```python
from build123d import *

# Parameters (mm, degrees)
EXTRUDE_1_DEPTH      = 5
EXTRUDE_1_DEPTH_BACK = 5


with BuildPart() as part:
    # 草图2 → 旋转1 (revolve)
    with BuildSketch(Plane.XY, mode=Mode.PRIVATE) as revolve_1_sk:
        with BuildLine():
            Line((6.5, 21.057334971), (6.5, 4.5))
            Line((6.5, 4.5), (5.633974596, 4))
            Line((5.633974596, 4), (0, 4))
            Line((0, 4), (0, 22.97165153))
            ThreePointArc((0, 22.97165153), (2.770599147, 22.808562355), (5.502930419, 22.321547438))
            ThreePointArc((5.502930419, 22.321547438), (6.220737367, 21.862378589), (6.5, 21.057334971))
        make_face()
    revolve(revolve_1_sk.sketch.rotate(Axis((0, 4, 0), (0, 1, 0)), 270), axis=Axis((0, 4, 0), (0, 1, 0)))

    # 草图1 → 凸台-拉伸1 (add, two sides: drawn at the far end of the back side and taken through both)
    with BuildSketch(Plane.XY.offset(-EXTRUDE_1_DEPTH_BACK)):
        with BuildLine():
            Line((-3.333333333, 5.5), (3.25, 5.5))
            Line((3.25, 5.5), (3.25, 10.326555972))
            ThreePointArc((3.25, 10.326555972), (4.489879958, 13.979124546), (7.697085729, 16.12211093))
            ThreePointArc((7.697085729, 16.12211093), (17.943826668, 18.039495945), (27.776457135, 21.502362282))
            ThreePointArc((27.776457135, 21.502362282), (29.380060021, 22.573855474), (30, 24.400139761))
            Line((30, 24.400139761), (30, 26))
            ThreePointArc((30, 26), (29.121320344, 28.121320344), (27, 29))
            Line((27, 29), (25.932943889, 29))
            Line((25.932943889, 29), (-3.333333333, 21.158124653))
            Line((-3.333333333, 21.158124653), (-3.333333333, 5.5))
        make_face()
    extrude(amount=EXTRUDE_1_DEPTH + EXTRUDE_1_DEPTH_BACK)

    # 草图3 → 切除-旋转1 (revolve, cut)
    with BuildSketch(Plane.XY, mode=Mode.PRIVATE) as cut_revolve_1_sk:
        Polygon((0, 28.156296), (4, 28.156296), (4, 17.156296), (5, 17.156296), (5, -2.643704), (0, -2.643704), align=None)
    revolve(cut_revolve_1_sk.sketch.rotate(Axis((0, -2.643704, 0), (0, 1, 0)), 270), axis=Axis((0, -2.643704, 0), (0, 1, 0)), mode=Mode.SUBTRACT)


solid = part.part
```
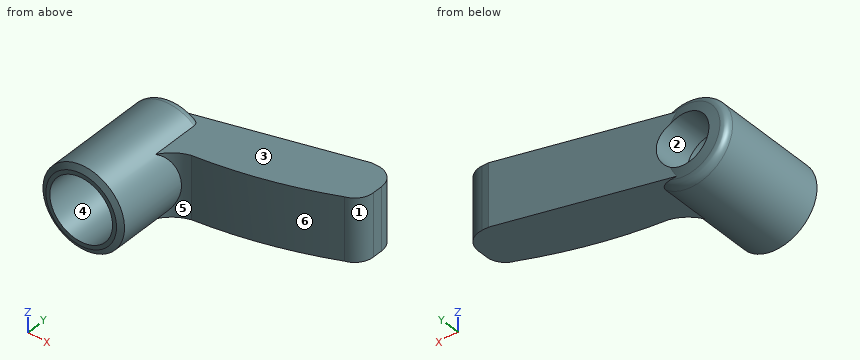
Input: part model. Units: mm. Frame: model coordinates. Face numbers are marked on the shaded views. A direction names the side the tool comes from. Coordinates: 2 decimals unless noted, no trailing zeros. Loops run counter-clockwise (first coordinate to the right, second up) from the corner with the lowest first, then second, coordinate; pieces in that order, holes last. Notation, with made-up numbers: (-40, 80) -> (-9, 80) arc R20 ccw to (-9, 93) -> close; hole circle Ø11 at (33.5, 75.5). An arc over 180 degrees is marked (long way). Use a Markdown table: item, result.
1) Cut plane C-C (z = 0). Return the cut outline in (x, y), then the cut area to 3 significant figures.
Results found:
| item | result |
|---|---|
| outline | (-6.5, 4.5) -> (-5.63, 4) -> (-5, 4) -> (-5, 17.16) -> (-4, 17.16) -> (-4, 22.63) arc R23.62 ccw to (-5.5, 22.32) arc R1.3 ccw to (-6.5, 21.06) -> close; (4, 17.16) -> (5, 17.16) -> (5, 4) -> (5.63, 4) -> (6.5, 4.5) -> (6.5, 15.66) arc R6 cw to (7.7, 16.12) arc R67.92 ccw to (27.78, 21.5) arc R3 ccw to (30, 24.4) -> (30, 26) arc R3 ccw to (27, 29) -> (25.93, 29) -> (4, 23.12) -> close |
| area | 261 mm2 |
2) Cut plane B-B (y = 10.5). Return the cut outline in (x, z).
Results found:
| item | result |
|---|---|
| outline | circle Ø13 at (0, 0); hole circle Ø10 at (0, 0) |
3) Pull-direction query (Z, two-part tool) for the marked faces 1, 2 and 3; classes: released by +Z, released by -Z, zero draft, split by the parting line, or undercut.
Results found:
| item | result |
|---|---|
| face 1 | zero draft |
| face 2 | undercut |
| face 3 | released by +Z |
4) Cut plane D-D (y = 14.25). Return the cut outline in (x, z), then the cut area to 3 significant figures.
Results found:
| item | result |
|---|---|
| outline | (4.15, -5) -> (4.71, -5) -> (4.71, -4.48) arc R6.5 ccw to (4.71, 4.48) -> (4.71, 5) -> (4.15, 5) arc R6.5 ccw (long way) to start; hole circle Ø10 at (0, 0) |
| area | 54.5 mm2 |
5) Cut plane A-A (x = 0). Return the cut outline in (y, z).
Results found:
| item | result |
|---|---|
| outline | (4, -5.63) -> (4.5, -6.5) -> (21.06, -6.5) arc R1.3 ccw to (22.32, -5.5) arc R23.62 ccw to (22.63, -4) -> (17.16, -4) -> (17.16, -5) -> (4, -5) -> close; (4, 5) -> (17.16, 5) -> (17.16, 4) -> (22.63, 4) arc R23.62 ccw to (22.32, 5.5) arc R1.3 ccw to (21.06, 6.5) -> (4.5, 6.5) -> (4, 5.63) -> close |
6) Access query for the marked faces 4, 5 and 6. Directions: +Z, -Z, +X, -X, +Y, -Y. A direction counts if a zero-diameter tool reaches every point of the face in a straight line with its end or side. Return the directions, or none.
Results found:
| item | result |
|---|---|
| face 4 | -Y |
| face 5 | +X, -Y |
| face 6 | +Z, -Z, +X, -Y |
7) Material intervals for line 1 along Z through (x, y) = (0, 11.5); line 2 along X through (y, z) = (20.85, 0), sorted ascending. Write a range as from..to.
Results found:
| item | result |
|---|---|
| line 1 | z = -6.5..-5, 5..6.5 |
| line 2 | x = -6.5..-4, 4..26.25 |
8) Contact query for flat-ended pins moving along their axis: pin 1 (5 mm diameter, centred on x = -2.5, z = 2, fed in from +Y); pin 2 (10 mm diameter, centred on x = 26, y = 24.5, fed in from -Z); pin 3 (2 mm diameter, centred on x = 20, z = 4.5, fed in from +Y); pin 4 (6.5 mm diameter, centred on x = 0, z = 0, fed in from -Y). Output: stop coordinate, or through.
Results found:
| item | result |
|---|---|
| pin 1 | stops at y = 22.63 |
| pin 2 | stops at z = -5 |
| pin 3 | stops at y = 27.68 |
| pin 4 | passes through |
